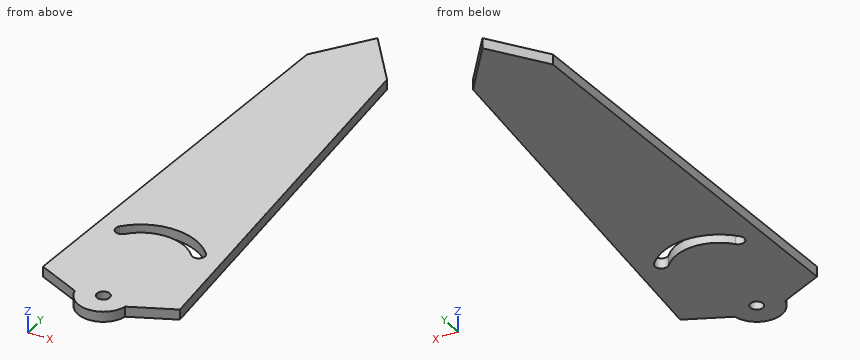
```python
from build123d import *

# Parameters (mm, degrees)
SKETCH2_R           = 5
BOSS_EXTRUDE1_DEPTH = 8
CUT_EXTRUDE1_DEPTH  = 10


with BuildPart() as part:
    # Sketch2 → Boss-Extrude1 (new body)
    with BuildSketch(Plane.XY):
        with BuildLine():
            Line((52.661413708, 1194.6), (30.792715617, 1507.336952872))
            Line((30.792715617, 1507.336952872), (0, 1548.052221237))
            Line((0, 1548.052221237), (-30.569888201, 1507.336952872))
            Line((-30.569888201, 1507.336952872), (-52.438586292, 1194.6))
            Line((-52.438586292, 1194.6), (-19.401690748, 1179.61379954))
            ThreePointArc((-19.401690748, 1179.61379954), (-0.057863528, 1164.108770521), (19.375843714, 1179.500995806))
            Line((19.375843714, 1179.500995806), (52.661413708, 1194.6))
        make_face()
        with Locations((0, 1184)):
            Circle(SKETCH2_R, mode=Mode.SUBTRACT)
    extrude(amount=BOSS_EXTRUDE1_DEPTH)

    # Sketch3 → Cut-Extrude1 (cut)
    with BuildSketch(Plane.XY.offset(8)):
        with BuildLine():
            ThreePointArc((33.346114696, 1262.714191316), (0.208267219, 1277.711712086), (-32.994808317, 1262.859158782))
            ThreePointArc((-32.994808317, 1262.859158782), (-32.584628739, 1255.799997875), (-25.525467832, 1256.210177452))
            ThreePointArc((-25.525467832, 1256.210177452), (0.186415379, 1267.711735961), (25.847787119, 1256.097917173))
            ThreePointArc((25.847787119, 1256.097917173), (32.905087979, 1255.656890456), (33.346114696, 1262.714191316))
        make_face()
    extrude(amount=-CUT_EXTRUDE1_DEPTH, mode=Mode.SUBTRACT)


solid = part.part
```
Geometry check sheet. Reference: the model listing, model coordinates, mm. Coordinates: 2 decimals unless noted, no trailing zeros. Order: outer loops, then holes, each group sorted by start corner. A loop starts at its lowest first (then second) coordinate and runs counter-clockwise, first axis right, second up. Notation, with made-up numbers: (-33, -15) - (-12, -15) arc R23 ccw to (-12, 17) - close; hole circle Ø9 at (27, 35.25). An arc over 180 degrees is marked (long way). Answer in a Markdown table with one row per item. Add a question column.
1. Section check A-A (x = -13.5). Enter the section's corners in (y, z), plus the area to 3 significant figures.
2. Material ranges on L1, parallel to Y at x = 0, z = 5.5; L2, parallel to Y at x = -3, z = 7.75; L3, parallel to X at y = 1184, z = 4.5, recorded low to high. Write a range as [from, to].
3. Gauge pin test, flat ends, axial feed: pin 1 Ø6 at (x, y) = (-9, 1477.5) entering from -Z; pin 2 Ø1 at (y, z) = (1486.5, 3.5) entering from +X; pin 3 Ø2 at (y, z) = (1430, 2.5) entering from +X; pin 4 Ø1 at (x, z) = (26.5, 1.5) entering from +Y. Record the tip position at first contact, or that the pin passes through.
4. Section check C-C (z = 3). Enter the section's corners in (x, y).
5. Section check B-B (y = 1184). Enter the section's corners in (x, z).
6. Section check D-D (y = 1388.5). Enter the section's corners in (x, z), plus the area to 3 significant figures.
Data:
| question | item | result |
|---|---|---|
| 1 | outline | (1169.39, 0) - (1264.9, 0) - (1264.9, 8) - (1169.39, 8) - close; (1275.57, 0) - (1530.07, 0) - (1530.07, 8) - (1275.57, 8) - close |
| 1 | area | 2,800 mm² |
| 2 | L1 | y = [1164.11, 1179], [1189, 1267.71], [1277.71, 1548.05] |
| 2 | L2 | y = [1164.34, 1180], [1188, 1267.57], [1277.6, 1544.06] |
| 2 | L3 | x = [-29.07, -5], [5, 29.29] |
| 3 | pin 1 | stops at z = 0 |
| 3 | pin 2 | stops at x = 32.28 |
| 3 | pin 3 | stops at x = 36.27 |
| 3 | pin 4 | stops at y = 1513.67 |
| 4 | outline | (-52.44, 1194.6) - (-19.4, 1179.61) arc R19.89 ccw to (19.38, 1179.5) - (52.66, 1194.6) - (30.79, 1507.34) - (0, 1548.05) - (-30.57, 1507.34) - close; hole (-32.99, 1262.86) arc R5 ccw to (-25.53, 1256.21) arc R34.32 cw to (25.85, 1256.1) arc R5 ccw to (33.35, 1262.71) arc R44.32 ccw to start; hole circle Ø10 at (0, 1184) |
| 5 | outline | (-29.07, 0) - (-5, 0) - (-5, 8) - (-29.07, 8) - close; (5, 0) - (29.29, 0) - (29.29, 8) - (5, 8) - close |
| 6 | outline | (-38.88, 0) - (39.1, 0) - (39.1, 8) - (-38.88, 8) - close |
| 6 | area | 624 mm² |
